from build123d import *

# Parameters (mm, degrees)
SKETCH_2_R          = 11.6
CUT_EXTRUDE_1_DEPTH = 3.5


with BuildPart() as part:
    # 草图1 → 旋转1 (revolve)
    with BuildSketch(Plane(origin=(0, 0, 0), x_dir=(0, 0, -1), z_dir=(1, 0, 0)), mode=Mode.PRIVATE) as revolve_1_sk:
        Polygon((-9.333333333, 0), (-9.333333333, 2.3865), (-8.719833333, 3), (18.5, 3), (18.5, 5.8), (21.791789368, 5.8), (22, 5.022947342), (22, 0), align=None)
    revolve(revolve_1_sk.sketch.rotate(Axis((0, 0, -22), (0, 0, 1)), 270), axis=Axis((0, 0, -22), (0, 0, 1)))

    # 草图2 → 切除-拉伸1 (cut)
    with BuildSketch(Plane(origin=(0, 0, -22), x_dir=(-1, 0, 0), z_dir=(0, 0, -1))):
        Circle(SKETCH_2_R)
        Polygon((0, -5.8), (5.022947342, -2.9), (5.022947342, 2.9), (0, 5.8), (-5.022947342, 2.9), (-5.022947342, -2.9), align=None, mode=Mode.SUBTRACT)
    extrude(amount=-CUT_EXTRUDE_1_DEPTH, mode=Mode.SUBTRACT)


solid = part.part
Verification items for the finished model (mm, model axes). A direction names the side the tool comes from. Coordinates: 2 decimals unless noted, no trailing zeros. Write each loop counter-clockwise with the first axis right and the second up, starting at its lowest first coordinate (ties: lowest second). Pieces come first, ordered by that corner, then holes. Notation, with made-up numbers: M 87,-35 L 115,-35 A26 ccw 115,-10 Z; hole C -15,-4 d1. An arc over 180 degrees is marked long. One line per question, with ' | ' between items.
1) Depth check by flat-ended pin: pin 1 Ø1 at (x, z) = (3, -12) entering from -Y; pin 2 Ø1.5 at (x, z) = (-2.5, -19) entering from -Y; pin 3 Ø5 at (x, z) = (1, -5) entering from +Y. Enter the tip coordinate at first touch or a pass-through.
Solutions:
pin 1: y = -1.66 | pin 2: y = -4.79 | pin 3: y = 3
2) Material ranges on L1, parallel to Y at x = 0, z = 0.5; L2, parallel to Z at x = 2.75, y = 2; L3, parallel to X at y = -2.75, z = -3, recorded low to high.
Solutions:
L1: -3 to 3 | L2: -22 to -18.5 | L3: -1.2 to 1.2
3) Sectioned sample at A-A on z = -10. Record the cut outline in (x, y).
Solutions:
outline: C 0,0 d6
4) Access from +Z, -Z, +X, -X, +Y, -Y to the whole of each face (thin tool, end or side, straight path). Record for faces 1 (the face through (0, 0, 9.333)), 2 (the face through (-2.2, -2.5, -18.5)).
Solutions:
face 1: +Z, +X, -X, +Y, -Y | face 2: +Z
